Answer from the drawing. Dimensions are ordinates in mm from the lowest x, y and z of the part. A direction names the side the tool comes from. Give positions to 0.01 mm unless a question says otherwise; leave off trailing zeros. Loops run counter-clockwise (first coordinate to the right, second up) from the corner with the lowest first, then second, coordinate; pieces in that order, holes last. Notation, with made-up numbers: (-22, 3) -> (31, 3) arc R33 ccw to (31, 35) -> close; hole circle Ø3 at (53.25, 37.25). An arc over 180 degrees is marked (long way). Write each question's results on one line, items separated by ' | '. Start each with the question number.
Item 1: Determine the mould class of the marked faces 3, 4, 5 and 6 for opening direction Y: +Y half, -Y half, draft (parallel to the pull), parting line (faces both ways), or undercut.
Item 2: Section D-D on z = 144.5 is taken. Write down the section's boundary in (x, y).
Item 3: Find the intervals of material crossed by line 1 (Y direction, x = 350, z = 17); line 2 (X direction, y = 200, z = 37.5); line 3 (X direction, y = 198.5, z = 56), in increasing order.
Item 4: Section A-A on z = 30 is taken. Write down the section's boundary in (x, y).
Item 5: Which of the six approach directions +Z, -Z, +X, -X, +Y, -Y give full straight-line access (tool end or side, diameter ignored) to the marked faces 1 and 2?
Item 6: Section C-C on y = 500 is taken. Write down the section's boundary in (x, z).
Item 7: Section B-B on x = 350 is taken. Write down the section's boundary in (y, z), and give its area (3 significant figures).
Item 8: Each of these flat-tipped pins is pushed along its axis until it touches: P1, Ø5, axis at x = 230, y = 110.5, coming from the +Z side; P2, Ø10, axis at x = 266, y = 280.5, coming from the -Z side; P3, Ø3, axis at y = 471, z = 95, coming from the -X side; P4, Ø1.5, axis at x = 166.5, z = 201.5, coming from the +Y side. Where does it stop, or does it pass through?
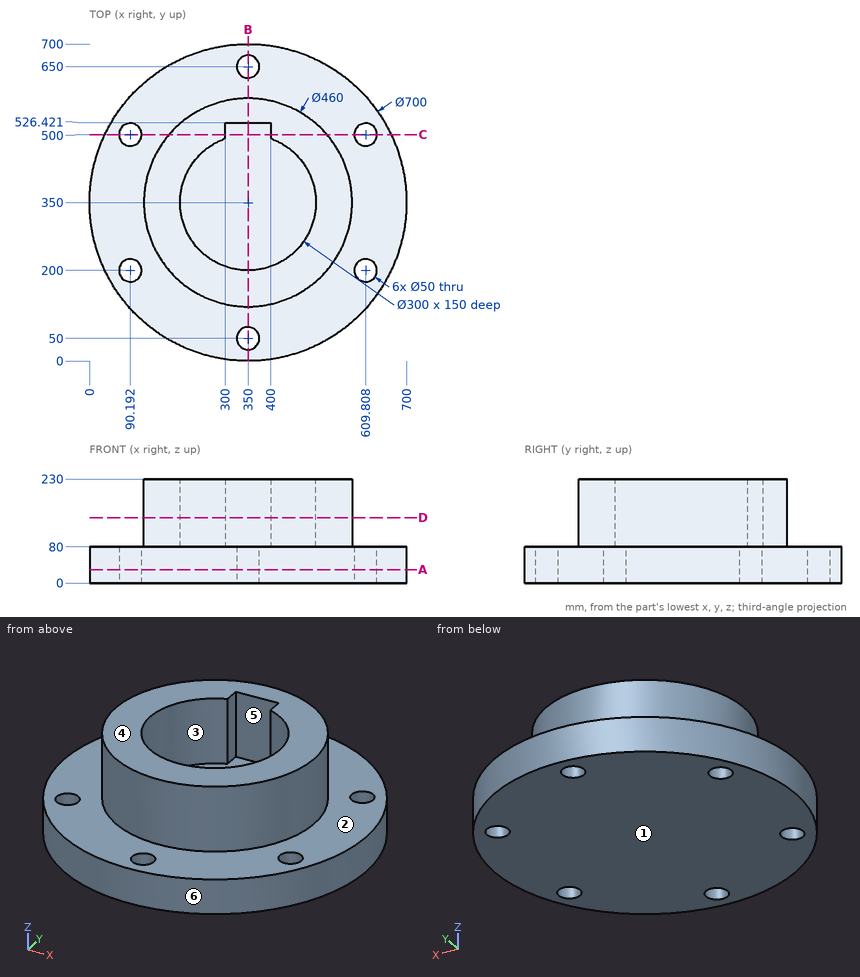
Findings:
1) face 3: undercut | face 4: draft | face 5: undercut | face 6: parting line
2) outline: circle Ø460 at (350, 350); hole (300, 491.42) arc R150 ccw (long way) to (400, 491.42) -> (400, 526.42) -> (300, 526.42) -> close
3) line 1: 0 to 25, 75 to 625, 675 to 700 | line 2: 33.77 to 65.19, 115.19 to 584.81, 634.81 to 666.23 | line 3: 34.49 to 65.24, 115.15 to 584.85, 634.76 to 665.51
4) outline: circle Ø700 at (350, 350); hole circle Ø50 at (90.19, 200); hole circle Ø50 at (90.19, 500); hole circle Ø50 at (350, 50); hole circle Ø50 at (350, 650); hole circle Ø50 at (609.81, 200); hole circle Ø50 at (609.81, 500)
5) face 1: -Z, +X, -X, +Y, -Y | face 2: +Z
6) outline: (33.77, 0) -> (65.19, 0) -> (65.19, 80) -> (33.77, 80) -> close; (115.19, 0) -> (584.81, 0) -> (584.81, 80) -> (524.36, 80) -> (524.36, 230) -> (400, 230) -> (400, 80) -> (300, 80) -> (300, 230) -> (175.64, 230) -> (175.64, 80) -> (115.19, 80) -> close; (634.81, 0) -> (666.23, 0) -> (666.23, 80) -> (634.81, 80) -> close
7) outline: (0, 0) -> (25, 0) -> (25, 80) -> (0, 80) -> close; (75, 0) -> (625, 0) -> (625, 80) -> (580, 80) -> (580, 230) -> (526.42, 230) -> (526.42, 80) -> (200, 80) -> (200, 230) -> (120, 230) -> (120, 80) -> (75, 80) -> close; (675, 0) -> (700, 0) -> (700, 80) -> (675, 80) -> close | area: 68,000 mm2
8) P1: z = 80 | P2: z = 0 | P3: x = 153.48 | P4: y = 489.65
